```python
from build123d import *

# Parameters (mm, degrees)
SKETCH_1_R                   = 3
EXTRUDE_1_DEPTH              = 25
HOLE_WIZARD_M8_1_D           = 9
HOLE_WIZARD_M8_1_CBORE_D     = 14
HOLE_WIZARD_M8_1_CBORE_DEPTH = 6
FILLET_1_R                   = 2


with BuildPart() as part:
    # 草图1 → 凸台-拉伸1 (new, symmetric)
    with BuildSketch(Plane(origin=(0, 0, 0), x_dir=(1, 0, 0), z_dir=(0, 1, 0))):
        with BuildLine():
            Line((10, -9), (10, -31))
            Line((10, -31), (0, -31))
            Line((0, -31), (0, 31))
            Line((0, 31), (10, 31))
            Line((10, 31), (10, 9))
            ThreePointArc((10, 9), (19, 0), (10, -9))
        make_face()
        with Locations(Location((10, 0, 0), (0, 0, 270))):
            Circle(SKETCH_1_R, mode=Mode.SUBTRACT)
    extrude(amount=EXTRUDE_1_DEPTH, both=True)

    # M8 六角凹头螺钉的柱形沉头孔1 (through all)
    with Locations(Plane(origin=(10, 0, 0), x_dir=(0, 0, -1), z_dir=(1, 0, 0))):
        with Locations((-20, 15), (-20, -15), (20, -15), (20, 15)):
            CounterBoreHole(HOLE_WIZARD_M8_1_D / 2, HOLE_WIZARD_M8_1_CBORE_D / 2, HOLE_WIZARD_M8_1_CBORE_DEPTH)

    # 圆角1
    fillet_1_edges = [part.edges().sort_by_distance(p)[0] for p in [
        (5, 25, -31),
        (5, -25, -31),
        (5, 25, 31),
        (5, -25, 31),
    ]]
    fillet(fillet_1_edges, radius=FILLET_1_R)


solid = part.part
```
Here's how the part is built. I have some questions about the finished solid (model axes, mm). A direction names the side the tool comes from. Coordinates: 2 decimals unless noted, no trailing zeros. Loops run counter-clockwise (first coordinate to the right, second up) from the corner with the lowest first, then second, coordinate; pieces in that order, holes last. Notation, with made-up numbers: (47, -9) -> (97, -9) arc R15 cw to (97, 3) -> close; hole circle Ø7 at (-26, 9). An arc over 180 degrees is marked (long way). Return JSON: item names as keys, results as strings.
1) Thinking about a two-plate mould opening in Z: for faces 1 (the face through (5, 25, 0)), 2 (the face through (7, -15, -13)), 3 (the face through (5.07, 24.43, -30.4)), 4 (the face through (4.93, -24.43, 30.4)), which applies, +Z half, -Z half, draft (parallel to the pull), parting line (faces both ways), or undercut?
Results below:
{"face 1": "draft", "face 2": "undercut", "face 3": "-Z half", "face 4": "+Z half"}
2) If we section it at B-B, the plane x = 3.25: Write out the boundary of the cut face in (y, z).
Results below:
{"outline": "(-25, -29) arc R2 ccw to (-23, -31) -> (23, -31) arc R2 ccw to (25, -29) -> (25, 29) arc R2 ccw to (23, 31) -> (-23, 31) arc R2 ccw to (-25, 29) -> close; hole circle Ø9 at (-15, -20); hole circle Ø9 at (-15, 20); hole circle Ø9 at (15, -20); hole circle Ø9 at (15, 20)"}
3) If we section it at C-C, the plane z = 0: Write out the boundary of the cut face in (x, y), then the cut area to 3 significant figures.
Results below:
{"outline": "(0, -25) -> (7, -25) -> (7, 25) -> (0, 25) -> close; (13, -25) -> (19, -25) -> (19, 25) -> (13, 25) -> close", "area": "650 mm²"}
4) I need wall thicknesses on line 1 (Y direction, x = 1.95, z = 20); line 2 (Y direction, x = 6.75, z = -15.5); line 3 (X direction, y = -8.5, z = 10.5). Which ranges of each line are inside material? Lowest first, please. Write a range as from..to.
Results below:
{"line 1": "-25..-19.5, -10.5..10.5, 19.5..25", "line 2": "-25..-20.36, -9.64..9.64, 20.36..25", "line 3": "0..10"}
5) For faces 5 (the face through (4, -20, -20)), 6 (the face through (10, 0, -20)), 7 (the face through (4.93, 24.43, 30.4)), which set-ups out of +Z, -Z, +X, -X, +Y, -Y let a thin tool reach every point of the face, with its end or its side?
Results below:
{"face 5": "+X", "face 6": "-Z, +X, +Y, -Y", "face 7": "+Z, +X, -X, +Y"}
6) Will these pins go through, and if not, where does the flat tip stop? pin 1 (11 mm diameter, centred on y = 17, z = -16.5, fed in from +X); pin 2 (7 mm diameter, centred on y = -15.5, z = -21, fed in from +X); pin 3 (4 mm diameter, centred on y = -14.5, z = 20, fed in from +X); pin 4 (24 mm diameter, centred on y = 0.5, z = -19.5, fed in from +X).
Results below:
{"pin 1": "x = 10", "pin 2": "x = 4", "pin 3": "through", "pin 4": "x = 14.97"}
7) If we section it at A-A, the plane y = -17: Write out the boundary of the cut face in (x, z), then the cut area to 3 significant figures.
Results below:
{"outline": "(0, -31) -> (10, -31) -> (10, -26.71) -> (4, -26.71) -> (4, -24.03) -> (0, -24.03) -> close; (0, -15.97) -> (4, -15.97) -> (4, -13.29) -> (10, -13.29) -> (10, -9) arc R9 ccw to (10, 9) -> (10, 13.29) -> (4, 13.29) -> (4, 15.97) -> (0, 15.97) -> close; (0, 24.03) -> (4, 24.03) -> (4, 26.71) -> (10, 26.71) -> (10, 31) -> (0, 31) -> close; hole circle Ø6 at (10, 0)", "area": "493 mm²"}
8) If we section it at D-D, the plane z = 20: Write out the boundary of the cut face in (x, y).
Results below:
{"outline": "(0, -25) -> (10, -25) -> (10, -22) -> (4, -22) -> (4, -19.5) -> (0, -19.5) -> close; (0, -10.5) -> (4, -10.5) -> (4, -8) -> (10, -8) -> (10, 8) -> (4, 8) -> (4, 10.5) -> (0, 10.5) -> close; (0, 19.5) -> (4, 19.5) -> (4, 22) -> (10, 22) -> (10, 25) -> (0, 25) -> close"}
